Can you work these out from the model? Positions are in its coordinate system, mm. A direction names the side the tool comes from. Coordinates: 2 decimals unless noted, no trailing zeros. Loops run counter-clockwise (first coordinate to the right, second up) from the corner with the lowest first, then second, coordinate; pieces in that order, holes last. Notation, with made-up numbers: (-2.5, 12.25) -> (39.5, 12.25) arc R26 ccw to (39.5, 37.25) -> close; hole circle Ø8 at (63, 48). An arc over 180 degrees is marked (long way). Put each result on its own line as item: value. Start each with the question number.
Item 1: For faces 4 (the cylindrical face through (4.88, 24.48, -1.08)), 5 (the cylindrical face through (9.9, 10.6, -9.9)), 6 (the cylindrical face through (-10.006, 15.972, 2.222)), which set-ups out of +Z, -Z, +X, -X, +Y, -Y let a thin tool reach every point of the face, with its end or its side?
Item 2: Will these pins go through, and if not, where does the flat tip stop? P1, Ø1, axis at x = 3.5, z = -5.5, coming from the +Y side; P2, Ø1.8, axis at x = 0, z = 0, coming from the -Y side; P3, Ø5, axis at x = -1, z = -0.5, coming from the -Y side.
Item 3: If we section it at C-C on y = 25: Please give me the cut outline in (x, z), plus the area to 3 significant figures.
Item 4: If we section it at B-B on y = 8: Please give me the cut outline in (x, z).
Item 5: Please list where these lines run through material, in increasing order: L1, parallel to X at y = 25.75, z = 0; L2, parallel to X at y = 4.75, z = 0; L3, parallel to Z at x = -5.75, y = 16.25. Write a range as from..to.
Item 6: We'd pull the mould along X, two halves only. Please class faces 1 (the cylindrical face through (-9.76, 7.41, 2.17)), 2 (the flat face through (0, 11, -12.5)), 3 (the flat face through (12.5, 11, 0)): pulls with the +X half, pulls with the -X half, needs draft (parallel to the pull), parting line crosses it, or undercut.
```python
from build123d import *

# Parameters (mm, degrees)
FILLET1_R           = 0.4
SKETCH2_R           = 10
CUT_EXTRUDE1_DEPTH  = 14
SKETCH3_R           = 10.25
CUT_EXTRUDE2_DEPTH  = 4
SKETCH4_R           = 1.5
CUT_EXTRUDE3_DEPTH  = 90
CHAMFER1_SIZE       = 0.3
CHAMFER2_SIZE       = 1
SKETCH5_OUTSIDE_W   = 39.586
SKETCH5_OUTSIDE_H   = 39.586
SKETCH5_OUTSIDE_W_2 = 25
SKETCH5_OUTSIDE_H_2 = 25
CUT_EXTRUDE4_DEPTH  = 90


with BuildPart() as part:
    # Sketch1 → Revolve1 (revolve)
    with BuildSketch(Plane.XY, mode=Mode.PRIVATE) as revolve1_sk:
        Polygon((0, 0), (-14, 0), (-14, 21), (-4.4, 21), (-4.4, 22.2), (-5, 22.2), (-5, 27), (0, 27), align=None)
    revolve(revolve1_sk.sketch.rotate(Axis((0, 27, 0), (0, -1, 0)), 270), axis=Axis((0, 27, 0), (0, -1, 0)))

    # Fillet1
    fillet1_edges = [part.edges().sort_by_distance(p)[0] for p in [
        (0, 22.2, -4.4),
        (0, 21, -4.4),
    ]]
    fillet(fillet1_edges, radius=FILLET1_R)

    # Sketch2 → Cut-Extrude1 (cut)
    with BuildSketch(Plane.XZ):
        with Locations(Location((0, 0, 0), (0, 0, 270))):
            Circle(SKETCH2_R)
    extrude(amount=-CUT_EXTRUDE1_DEPTH, mode=Mode.SUBTRACT)

    # Sketch3 → Cut-Extrude2 (cut)
    with BuildSketch(Plane.XZ.offset(-14)):
        with Locations(Location((0, 0, 0), (0, 0, 270))):
            Circle(SKETCH3_R)
    extrude(amount=-CUT_EXTRUDE2_DEPTH, mode=Mode.SUBTRACT)

    # Sketch4 → Cut-Extrude3 (cut)
    with BuildSketch(Plane.XZ.offset(-18)):
        with Locations(Location((0, 0, 0), (0, 0, 270))):
            Circle(SKETCH4_R)
    extrude(amount=-CUT_EXTRUDE3_DEPTH, mode=Mode.SUBTRACT)

    # Chamfer1
    chamfer1_edges = [part.edges().sort_by_distance(p)[0] for p in [
        (0, 27, -5),
    ]]
    chamfer(chamfer1_edges, length=CHAMFER1_SIZE)

    # Chamfer2
    chamfer2_edges = [part.edges().sort_by_distance(p)[0] for p in [
        (0, 0, 10),
    ]]
    chamfer(chamfer2_edges, length=CHAMFER2_SIZE)

    # Sketch5 outside → Cut-Extrude4 (cut)
    with BuildSketch(Plane(origin=(0, 21, 0), x_dir=(1, 0, 0), z_dir=(0, 1, 0))):
        Rectangle(SKETCH5_OUTSIDE_W, SKETCH5_OUTSIDE_H)
        Rectangle(SKETCH5_OUTSIDE_W_2, SKETCH5_OUTSIDE_H_2, mode=Mode.SUBTRACT)
    extrude(amount=-CUT_EXTRUDE4_DEPTH, mode=Mode.SUBTRACT)


solid = part.part
```
Solutions:
1. face 4: +Y
1. face 5: -Z, +X, +Y, -Y
1. face 6: none
2. P1: y = 21
2. P2: through
2. P3: y = 18
3. outline: circle Ø10 at (0, 0); hole circle Ø3 at (0, 0)
3. area: 71.5 mm^2
4. outline: (-12.5, -6.3) arc R14 ccw to (-6.3, -12.5) -> (6.3, -12.5) arc R14 ccw to (12.5, -6.3) -> (12.5, 6.3) arc R14 ccw to (6.3, 12.5) -> (-6.3, 12.5) arc R14 ccw to (-12.5, 6.3) -> close; hole circle Ø20 at (0, 0)
5. L1: -5..-1.5, 1.5..5
5. L2: -12.5..-10, 10..12.5
5. L3: -12.5..-8.49, 8.49..12.5
6. face 1: undercut
6. face 2: needs draft
6. face 3: pulls with the +X half
